Part model, mm, in its own coordinate system. A direction names the side the tool comes from. Give positions to 0.01 mm unless a question says otherwise; leave off trailing zeros. Order: outer loops, then holes, each group sorted by start corner. A loop starts at its lowest first (then second) coordinate and runs counter-clockwise, first axis right, second up.
from build123d import *

# Parameters (mm, degrees)
CUT_EXTRUDE1_START    = -10
CUT_EXTRUDE1_DEPTH    = 10
M3_TAPPED_HOLE1_D     = 2.5
M3_TAPPED_HOLE1_DEPTH = 7.5
M3_TAPPED_HOLE1_TIP   = 0.751075774


with BuildPart() as part:
    # Sketch1 → Revolve1 (revolve)
    with BuildSketch(Plane.XY, mode=Mode.PRIVATE) as revolve1_sk:
        Polygon((-5, 0), (-9, 0), (-9, -8), (-25, -8), (-25, -9), (-22, -9), (-22, -13), (-25, -13), (-25, -14), (-5, -14), align=None)
    revolve(revolve1_sk.sketch.rotate(Axis((0, 0, 0), (0, -1, 0)), 270), axis=Axis((0, 0, 0), (0, -1, 0)))

    # Sketch2 → Cut-Extrude1 (cut)
    with BuildSketch(Plane(origin=(0, -13, 0), x_dir=(1, 0, 0), z_dir=(0, 1, 0)).offset(CUT_EXTRUDE1_START)):
        with BuildLine():
            Line((-1, -21.977260976), (-1, -40))
            Line((-1, -40), (1, -40))
            Line((1, -40), (1, -21.977260976))
            ThreePointArc((1, -21.977260976), (0, -22), (-1, -21.977260976))
        make_face()
    extrude(amount=CUT_EXTRUDE1_DEPTH, mode=Mode.SUBTRACT)

    # M3 Tapped Hole1
    with Locations(Plane(origin=(0, -4, 9), x_dir=(1, 0, 0), z_dir=(0, 0, 1))):
        with Locations((0, 0)):
            Hole(M3_TAPPED_HOLE1_D / 2, depth=M3_TAPPED_HOLE1_DEPTH)
            with Locations((0, 0, -(M3_TAPPED_HOLE1_DEPTH + M3_TAPPED_HOLE1_TIP / 2))):  # 118° drill point
                Cone(0, M3_TAPPED_HOLE1_D / 2, M3_TAPPED_HOLE1_TIP, mode=Mode.SUBTRACT)


solid = part.part
Item 1: Band-saw the part on B-B on z = 0. List the corners of the cut face in (x, y), plus the area to 3 significant figures.
Item 2: Band-saw the part on C-C on y = -10.25. List the corners of the cut face in (x, z), plus the area to 3 significant figures.
Item 3: Band-saw the part on A-A on x = 0. List the corners of the cut face in (y, z).
Item 4: Drill centre lines: probe 1 along Y at (x, z) = (-22, 7.5); probe 2 along Y at (x, z) = (-18, 1); probe 3 along X at (y, z) = (-6, 0). Where is each one in solid material? Low to high.
Item 5: Which spindle directions (+Z, -Z, +X, -X, +Y, -Y) get a long thin tool onto all of the face, cutting with end or side? Do faces 1 (the face through (22.1, -9, 1.7)), 2 (the face through (0.27, -5.22, 6.89)), 3 (the face through (11, -8, 0)). Say none if no direction does.
Item 6: Band-saw the part on D-D on z = 17. List the corners of the cut face in (x, y).
Item 7: Pull direction Z, two halves, no side cores. Call faces 4 (the face through (4.88, -6.9, -1.08)), 5 (the face through (-7.509, -8.507, 23.846)), 6 (the face through (17, -13, -15)): released by +Z, released by -Z, zero draft, split by the parting line, or undercut.
Item 8: Drop flat-ended pins along their axis: P1, Ø1, axis at x = -0.5, y = -6, coming from the +Z side; P2, Ø6, axis at x = 19.5, z = 13.5, coming from the +Y side; P3, Ø2, axis at x = 0, y = -4, coming from the -Z side. Give the stop position or say it passes through.
Working result:
1. outline: (-25, -14) - (-5, -14) - (-5, 0) - (-9, 0) - (-9, -8) - (-25, -8) - (-25, -9) - (-22, -9) - (-22, -13) - (-25, -13) - close; (5, -14) - (25, -14) - (25, -13) - (22, -13) - (22, -9) - (25, -9) - (25, -8) - (9, -8) - (9, 0) - (5, 0) - close
1. area: 280 mm2
2. outline: circle Ø44 at (0, 0); hole circle Ø10 at (0, 0)
2. area: 1,440 mm2
3. outline: (-14, -25) - (-13, -25) - (-13, -22) - (-9, -22) - (-9, -25) - (-8, -25) - (-8, -9) - (0, -9) - (0, -5) - (-14, -5) - close; (-14, 5) - (-5.25, 5) - (-5.25, 9) - (-8, 9) - (-8, 25) - (-9, 25) - (-9, 22) - (-14, 22) - close; (-2.75, 5) - (0, 5) - (0, 9) - (-2.75, 9) - close
4. probe 1: y = -14 to -13, -9 to -8
4. probe 2: y = -14 to -8
4. probe 3: x = -9 to -5, 5 to 9
5. face 1: none
5. face 2: +Z
5. face 3: +Y
6. outline: (-18.33, -14) - (18.33, -14) - (18.33, -13) - (13.96, -13) - (13.96, -9) - (18.33, -9) - (18.33, -8) - (-18.33, -8) - (-18.33, -9) - (-13.96, -9) - (-13.96, -13) - (-18.33, -13) - close
7. face 4: undercut
7. face 5: split by the parting line
7. face 6: zero draft
8. P1: stops at z = 9
8. P2: stops at y = -8
8. P3: stops at z = -9
